Verification items for the finished model (mm, model axes). Face numbers are marked on the shaded views. A direction names the side the tool comes from. Give positions to 0.01 mm unless a question says otherwise; leave off trailing zeros. Order: outer loops, then holes, each group sorted by start corner. A loop starts at its lowest first (then second) coordinate and runs counter-clockwise, first axis right, second up. Notation, with made-up numbers: M -40,84.5 L 9,84.5 A12 cw 9,94.5 Z; hole C 49.25,83.5 d8. An arc over 180 degrees is marked long. Answer as a JSON object with one key per item and string values.
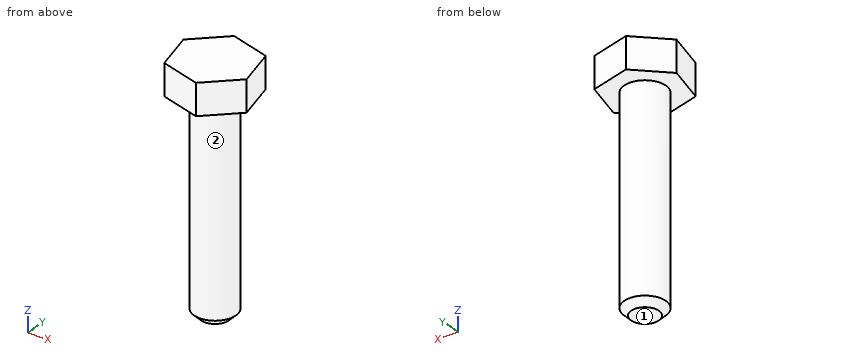
```python
from build123d import *

# Parameters (mm, degrees)
SKETCH1_R           = 6
BOSS_EXTRUDE1_DEPTH = 4.5
SKETCH2_OUTSIDE_W   = 17.512
SKETCH2_OUTSIDE_H   = 17.512
CUT_EXTRUDE1_DEPTH  = 4.5
SKETCH3_R           = 3
BOSS_EXTRUDE2_DEPTH = 30
CHAMFER1_SIZE       = 1


with BuildPart() as part:
    # Sketch1 → Boss-Extrude1 (new body)
    with BuildSketch(Plane.XY):
        Circle(SKETCH1_R)
    extrude(amount=BOSS_EXTRUDE1_DEPTH)

    # Sketch2 outside → Cut-Extrude1 (cut)
    with BuildSketch(Plane(origin=(0, 0, 0), x_dir=(-1, 0, 0), z_dir=(0, 0, -1))):
        Rectangle(SKETCH2_OUTSIDE_W, SKETCH2_OUTSIDE_H)
        Polygon((4.317619028, -4.16631323), (5.766942611, 1.656011147), (1.449323583, 5.822324377), (-4.317619028, 4.16631323), (-5.766942611, -1.656011147), (-1.449323583, -5.822324377), align=None, mode=Mode.SUBTRACT)
    extrude(amount=-CUT_EXTRUDE1_DEPTH, mode=Mode.SUBTRACT)

    # Sketch3 → Boss-Extrude2 (add)
    with BuildSketch(Plane(origin=(0, 0, 0), x_dir=(-1, 0, 0), z_dir=(0, 0, -1))):
        Circle(SKETCH3_R)
    extrude(amount=BOSS_EXTRUDE2_DEPTH)

    # Chamfer1
    chamfer1_edges = [part.edges().sort_by_distance(p)[0] for p in [
        (3, 0, -30),
    ]]
    chamfer(chamfer1_edges, length=CHAMFER1_SIZE)


solid = part.part
```
Q1. Section check D-D on y = -5. Record the cut outline in (x, z).
Resolved:
{"outline": "M -1.41,0 L 2.3,0 L 2.3,4.5 L -1.41,4.5 Z"}
Q2. Section check B-B on x = 0. Record the cut outline in (y, z), then the cut area to 3 significant figures.
Resolved:
{"outline": "M -5.41,0 L -3,0 L -3,-29 L -2,-30 L 2,-30 L 3,-29 L 3,0 L 5.41,0 L 5.41,4.5 L -5.41,4.5 Z", "area": "228 mm²"}
Q3. Material ranges on L1, parallel to Z at x = 4.25, y = -3; L2, parallel to Y at x = 0, z = -10; L3, parallel to X at y = -0.75, z = -18, recorded low to high.
Resolved:
{"L1": "z = 0 to 4.5", "L2": "y = -3 to 3", "L3": "x = -2.9 to 2.9"}
Q4. Section check C-C on z = -20.5. Record the cut outline in (x, y), then the cut area to 3 significant figures.
Resolved:
{"outline": "C 0,0 d6", "area": "28.3 mm²"}
Q5. Tool access check on the marked faces 1 and 2. Record the directions out of +Z, -Z, +X, -X, +Y, -Y that give a thin tool (end or side, any length) a straight path to the whole face; none if there is none.
Resolved:
{"face 1": "-Z, +X, -X, +Y, -Y", "face 2": "-Z"}
Q6. Section check A-A on y = 0. Record the cut outline in (x, z).
Resolved:
{"outline": "M -5.35,0 L -3,0 L -3,-29 L -2,-30 L 2,-30 L 3,-29 L 3,0 L 5.35,0 L 5.35,4.5 L -5.35,4.5 Z"}
Q7. Gauge pin test, flat ends, axial feed: pin 1 Ø6 at (y, z) = (-1, -4) entering from -X; pin 2 Ø3 at (x, z) = (1.5, -0.5) entering from -Y; pin 3 Ø3 at (x, z) = (-3.5, -22.5) entering from +Y; pin 4 Ø3 at (y, z) = (-1.5, -9.5) entering from +X. Record the tip position at first contact, or that the pin passes through.
Resolved:
{"pin 1": "stops at x = -3", "pin 2": "stops at y = -5.82", "pin 3": "stops at y = 2.24", "pin 4": "stops at x = 3"}
